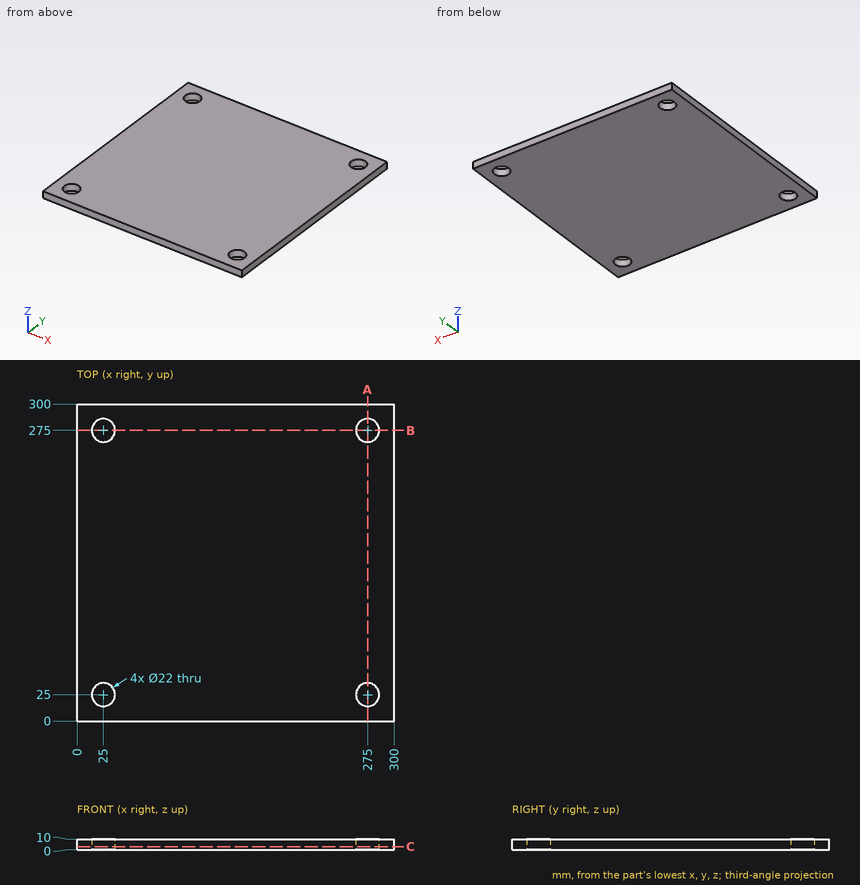
Print and shaded views of the part. All mm, measured from the part's lowest x, y and z. Give positions to 0.01 mm unless a question says otherwise; leave off trailing zeros. Order: outer loops, then holes, each group sorted by start corner. A loop starts at its lowest first (then second) coordinate and runs counter-clockwise, first axis right, second up. Notation, with made-up numbers: (-21, 16.5) - (34, 16.5) arc R35 ccw to (34, 50.5) - close; hole circle Ø4 at (1.5, 12). An arc over 180 degrees is marked (long way). One line per item, written item: value.
Item 1: Slice it at A-A (x = 275). List the corners of the cut face in (y, z).
Response values:
outline: (0, 0) - (14, 0) - (14, 10) - (0, 10) - close; (36, 0) - (264, 0) - (264, 10) - (36, 10) - close; (286, 0) - (300, 0) - (300, 10) - (286, 10) - close
Item 2: Wall check: line 1 (Y direction, x = 25, z = 4); line 2 (X direction, y = 266, z = 6.5). Give the ranges that are in metal, low to high.
Response values:
line 1: 0 to 14, 36 to 264, 286 to 300
line 2: 0 to 18.68, 31.32 to 268.68, 281.32 to 300
Item 3: Pin check, flat tip, straight feed: pin 1 Ø13 at (x, y) = (275, 25) entering from -Z. Stop position of the tip, or through.
Response values:
pin 1: through
Item 4: Slice it at C-C (z = 2.75). List the corners of the cut face in (x, y), then the cut area to 3 significant figures.
Response values:
outline: (0, 0) - (300, 0) - (300, 300) - (0, 300) - close; hole circle Ø22 at (25, 25); hole circle Ø22 at (25, 275); hole circle Ø22 at (275, 25); hole circle Ø22 at (275, 275)
area: 88,500 mm2
